The listing builds one solid part. Answer for the finished solid, in the listing's coordinates (mm). A direction names the side the tool comes from. Coordinates: 2 decimals unless noted, no trailing zeros. Order: outer loops, then holes, each group sorted by start corner. A loop starts at its lowest first (then second) coordinate and runs counter-clockwise, first axis right, second up. Notation, with made-up numbers: (11, 70.25) - (18, 70.25) arc R12 ccw to (18, 83.25) - close; hole circle Ø4 at (78.25, 86.5). An arc over 180 degrees is marked (long way). Use one line per item in the form item = value. Start each with the question number.
Item 1: A tool of negligible diameter and unlimited length cuts with its end or side. For faces 1 (the cylindrical face through (18.284, 17.683, -24.453)), 2 (the cylindrical face through (-18.28, 7.54, -15.78)), 3 (the cylindrical face through (-19.349, 2.81, 35.043)), from which of +Z, -Z, +X, -X, +Y, -Y can it reach the whole face along a straight path? Write none if from no direction.
Item 2: Section C-C, the plane z = 0 is taken. Write down the section's boundary in (x, y), and give its area (3 significant figures).
Item 3: Each of these flat-tipped pins is pushed along its axis until it touches: pin 1 Ø5.5 at (x, z) = (20, 17) entering from +Y; pin 2 Ø3.5 at (x, z) = (20, 40) entering from -Y; pin 3 Ø11.5 at (x, z) = (-20, 40) entering from +Y; pin 4 Ø3 at (x, z) = (-20.5, 38.5) entering from -Y. Where does it stop, or does it pass through?
Item 4: The mould has two halves that part along X. Classify faces 4 (the flat face through (30, 10, 1)), 5 (the cylindrical face through (20.651, 2.81, -44.957)), 6 (the flat face through (-14, 0, -12)): released by +X, released by -X, zero draft, split by the parting line, or undercut.
Item 5: Section B-B, the plane y = 18.5 is taken. Count the separate pieces of the cut face and the enclosed holes in it, and give its area (3 significant figures).
Item 6: Consider line 1 along X through (y, z) = (18.2, 19); line 2 along X through (y, z) = (2.25, -40); line 3 along Z through (x, y) = (-20, 12.5). Determine where each line is inside the solid, lowest interval first. Write a range as [from, to].
Item 7: Section A-A, the plane z = 19 is taken. Write down the section's boundary in (x, y).
Item 8: Section D-D, the plane x = 2 is taken. Write down the section's boundary in (y, z), and give its area (3 significant figures).
from build123d import *

# Parameters (mm, degrees)
SKETCH_1_W                  = 60
SKETCH_1_H                  = 100
EXTRUDE_1_DEPTH             = 20
SKETCH_2_R                  = 17.75
CUT_EXTRUDE_1_DEPTH         = 20
HOLE_WIZARD_1_D             = 6.6
HOLE_WIZARD_1_DEPTH         = 30
HOLE_WIZARD_1_CBORE_D       = 11
HOLE_WIZARD_1_CBORE_DEPTH   = 4.7
HOLE_WIZARD_1_TIP           = 1.982840043
CHAMFER_1_SIZE              = 5
HOLE_WIZARD_1_2_D           = 5.5
HOLE_WIZARD_1_2_DEPTH       = 30
HOLE_WIZARD_1_2_CBORE_D     = 10
HOLE_WIZARD_1_2_CBORE_DEPTH = 5.7
HOLE_WIZARD_1_2_TIP         = 1.652366702


with BuildPart() as part:
    # 草图1 → 凸台-拉伸1 (new body)
    with BuildSketch(Plane(origin=(0, 0, 0), x_dir=(1, 0, 0), z_dir=(0, 1, 0))):
        Rectangle(SKETCH_1_W, SKETCH_1_H)
    extrude(amount=EXTRUDE_1_DEPTH)

    # 草图2 → 切除-拉伸1 (cut)
    with BuildSketch(Plane(origin=(0, 20, 0), x_dir=(1, 0, 0), z_dir=(0, 1, 0))):
        with Locations(Location((0, 0, 0), (0, 0, 270))):
            Circle(SKETCH_2_R)
    extrude(amount=-CUT_EXTRUDE_1_DEPTH, mode=Mode.SUBTRACT)

    # Hole Wizard 1
    with Locations(Plane(origin=(0, 20, 0), x_dir=(1, 0, 0), z_dir=(0, 1, 0))):
        with Locations((19, 19), (19, -19), (-19, 19), (-19, -19)):
            CounterBoreHole(HOLE_WIZARD_1_D / 2, HOLE_WIZARD_1_CBORE_D / 2, HOLE_WIZARD_1_CBORE_DEPTH, depth=HOLE_WIZARD_1_DEPTH)
            with Locations((0, 0, -(HOLE_WIZARD_1_DEPTH + HOLE_WIZARD_1_TIP / 2))):  # 118° drill point
                Cone(0, HOLE_WIZARD_1_D / 2, HOLE_WIZARD_1_TIP, mode=Mode.SUBTRACT)

    # 倒角1
    chamfer_1_edges = [part.edges().sort_by_distance(p)[0] for p in [
        (30, 10, 50),
        (-30, 10, 50),
        (-30, 10, -50),
        (30, 10, -50),
    ]]
    chamfer(chamfer_1_edges, length=CHAMFER_1_SIZE)

    # Hole Wizard 1 2
    with Locations(Plane(origin=(0, 0, 0), x_dir=(-1, 0, 0), z_dir=(0, -1, 0))):
        with Locations((20, 40), (-20, 40), (20, -40), (-20, -40)):
            CounterBoreHole(HOLE_WIZARD_1_2_D / 2, HOLE_WIZARD_1_2_CBORE_D / 2, HOLE_WIZARD_1_2_CBORE_DEPTH, depth=HOLE_WIZARD_1_2_DEPTH)
            with Locations((0, 0, -(HOLE_WIZARD_1_2_DEPTH + HOLE_WIZARD_1_2_TIP / 2))):  # 118° drill point
                Cone(0, HOLE_WIZARD_1_2_D / 2, HOLE_WIZARD_1_2_TIP, mode=Mode.SUBTRACT)


solid = part.part
Response:
q1.face_1 = +Y
q1.face_2 = +Y, -Y
q1.face_3 = -Y
q2.outline = (-30, 0) - (-17.75, 0) - (-17.75, 20) - (-30, 20) - close; (17.75, 0) - (30, 0) - (30, 20) - (17.75, 20) - close
q2.area = 490 mm2
q3.pin_1 = 15.3
q3.pin_2 = through
q3.pin_3 = 20
q3.pin_4 = 5.7
q4.face_4 = released by +X
q4.face_5 = undercut
q4.face_6 = zero draft
q5.separate_pieces = 1
q5.enclosed_holes = 9
q5.area = 4,490 mm2
q6.line_1 = [-30, -24.5], [-13.5, 13.5], [24.5, 30]
q6.line_2 = [-30, -25], [-15, 15], [25, 30]
q6.line_3 = [-50, -42.75], [-37.25, -22.14], [-15.86, 15.86], [22.14, 37.25], [42.75, 50]
q7.outline = (-30, 0) - (-22.3, 0) - (-22.3, 15.3) - (-24.5, 15.3) - (-24.5, 20) - (-30, 20) - close; (-15.7, 0) - (15.7, 0) - (15.7, 15.3) - (13.5, 15.3) - (13.5, 20) - (-13.5, 20) - (-13.5, 15.3) - (-15.7, 15.3) - close; (22.3, 0) - (30, 0) - (30, 20) - (24.5, 20) - (24.5, 15.3) - (22.3, 15.3) - close
q8.outline = (0, -50) - (20, -50) - (20, -17.64) - (0, -17.64) - close; (0, 17.64) - (20, 17.64) - (20, 50) - (0, 50) - close
q8.area = 1,290 mm2
